The drawing under review shows one solid part. Ordinate dimensions are in mm from its lowest x, y, z. A direction names the side the tool comes from. Coordinates: 2 decimals unless noted, no trailing zeros. Loops run counter-clockwise (first coordinate to the right, second up) from the corner with the lowest first, then second, coordinate; pieces in that order, holes last. Notation, with made-up numbers: (-34, -14) -> (1, -14) arc R18 ccw to (1, -4) -> close; hole circle Ø1 at (-6.5, 52). An arc over 180 degrees is marked (long way). Use a Markdown table: item, result.
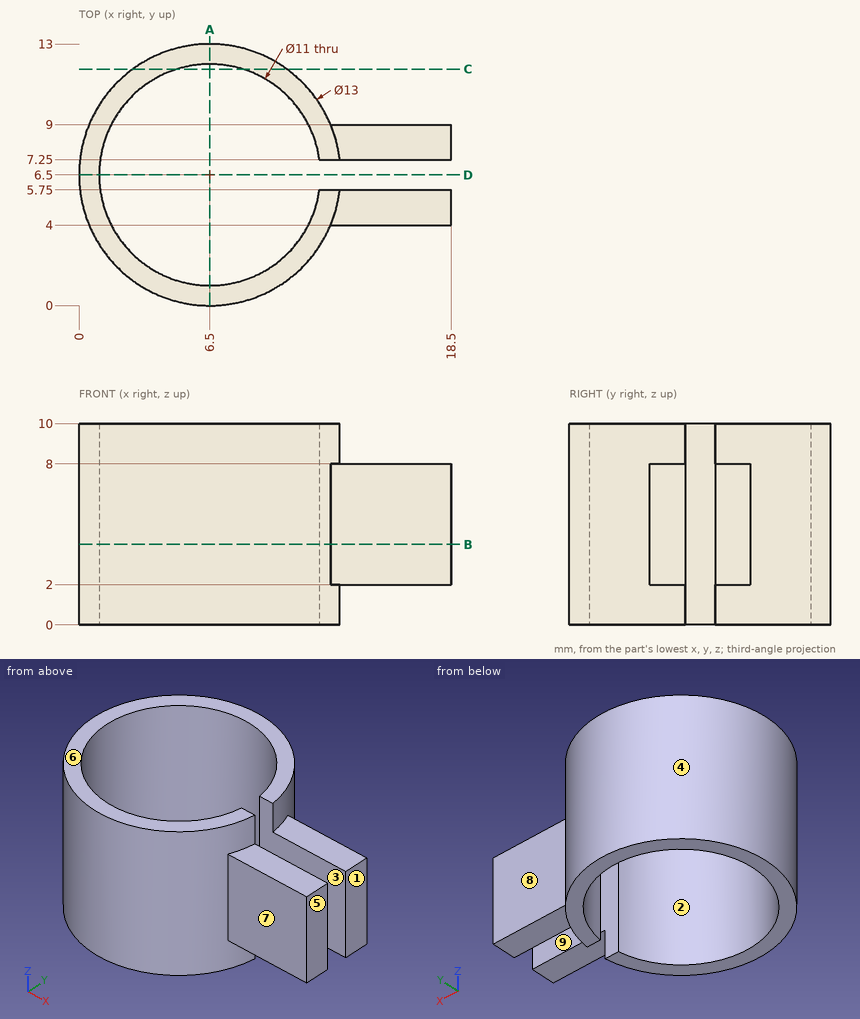
(1) For pin 1 Ø0.5 at (x, y) = (14.5, 5) entering from +Z; pin 2 Ø3.5 at (x, z) = (15, 4.5) entering from +Y; pin 3 Ø2 at (x, z) = (9, 8.5) entering from +Y, all flat-tipped, find the tip position at first contact; note any pin that passes through.
Found:
| item | result |
|---|---|
| pin 1 | stops at z = 8 |
| pin 2 | stops at y = 9 |
| pin 3 | stops at y = 12.82 |
(2) Take a section at B-B on z = 4. Write out the cut boundary in (x, y), plus the area to 3 significant figures.
Found:
| item | result |
|---|---|
| outline | (11.95, 5.75) arc R5.5 cw (long way) to (11.95, 7.25) -> (18.5, 7.25) -> (18.5, 9) -> (12.5, 9) arc R6.5 ccw (long way) to (12.5, 4) -> (18.5, 4) -> (18.5, 5.75) -> close |
| area | 56.2 mm^2 |
(3) Take a section at A-A on x = 6.5. Write out the cut boundary in (y, z), plus the area to 3 significant figures.
Found:
| item | result |
|---|---|
| outline | (0, 0) -> (1, 0) -> (1, 10) -> (0, 10) -> close; (12, 0) -> (13, 0) -> (13, 10) -> (12, 10) -> close |
| area | 20.0 mm^2 |
(4) Take a section at C-C on y = 11.75. Write out the cut boundary in (x, z).
Found:
| item | result |
|---|---|
| outline | (2.67, 0) -> (4.86, 0) -> (4.86, 10) -> (2.67, 10) -> close; (8.14, 0) -> (10.33, 0) -> (10.33, 10) -> (8.14, 10) -> close |
(5) For line 1 along Y through (x, z) = (15, 4.5); line 2 along Y through (x, z) = (6.5, 4.25); line 3 along X through (y, z) = (11.5, 4.5), list the stretches that pass through material, from the lowest coordinate up.
Found:
| item | result |
|---|---|
| line 1 | y = 4 to 5.75, 7.25 to 9 |
| line 2 | y = 0 to 1, 12 to 13 |
| line 3 | x = 2.35 to 4.21, 8.79 to 10.65 |
(6) Mouldability with a two-part tool opening along X and no side actions: class the marked faces 1, 2, 3 and 4 as pulls with the +X half, pulls with the -X half, needs draft (parallel to the pull), parting line crosses it, or undercut.
Found:
| item | result |
|---|---|
| face 1 | pulls with the +X half |
| face 2 | undercut |
| face 3 | needs draft |
| face 4 | parting line crosses it |
(7) For the marked faces 5, 6, 7, 8 and 9, list the 3-axis set-ups (+Z, -Z, +X, -X, +Y, -Y) from which the entire face can be reached by the end or side of a thin tool; tool diameter is ignored.
Found:
| item | result |
|---|---|
| face 5 | +Z, -Z, +X, +Y, -Y |
| face 6 | +Z, +X, -X, +Y, -Y |
| face 7 | +Z, -Z, +X, -Y |
| face 8 | +Z, -Z, +X, +Y |
| face 9 | +Z, -Z, +X |
(8) Take a section at D-D on y = 6.5. Write out the cut boundary in (x, z), plus the area to 3 significant figures.
Found:
| item | result |
|---|---|
| outline | (0, 0) -> (1, 0) -> (1, 10) -> (0, 10) -> close |
| area | 10.0 mm^2 |
